from build123d import *

# Parameters (mm, degrees)
SKETCH_2_W          = 55
SKETCH_2_H          = 61
EXTRUDE_1_DEPTH     = 3
SKETCH_3_R          = 1.6
CUT_EXTRUDE_1_DEPTH = 3
FILLET_1_R          = 5
CUT_EXTRUDE_2_DEPTH = 3
FILLET_2_R          = 2


with BuildPart() as part:
    # 草图2 → 凸台-拉伸1 (new body)
    with BuildSketch(Plane(origin=(0, 0, 0), x_dir=(0, 0, -1), z_dir=(1, 0, 0))):
        with Locations((27.5, 30.5)):
            Rectangle(SKETCH_2_W, SKETCH_2_H)
    extrude(amount=EXTRUDE_1_DEPTH)

    # 草图3 → 切除-拉伸1 (cut)
    with BuildSketch(Plane.ZY):
        with Locations((-5, 56)):
            Circle(SKETCH_3_R)
        with Locations((-5, 37.5)):
            Circle(SKETCH_3_R)
        with Locations((-50, 56)):
            Circle(SKETCH_3_R)
        with Locations((-50, 37.5)):
            Circle(SKETCH_3_R)
        with Locations((-37.5, 3)):
            Circle(SKETCH_3_R)
        with Locations((-17.5, 3)):
            Circle(SKETCH_3_R)
    extrude(amount=-CUT_EXTRUDE_1_DEPTH, mode=Mode.SUBTRACT)

    # 圆角1
    fillet_1_edges = [part.edges().sort_by_distance(p)[0] for p in [
        (1.5, 61, 0),
        (1.5, 61, -55),
        (1.5, 0, -55),
        (1.5, 0, 0),
    ]]
    fillet(fillet_1_edges, radius=FILLET_1_R)

    # 草图4 → 切除-拉伸2 (cut)
    with BuildSketch(Plane.ZY):
        Polygon((-39.417495765, 57), (-27.5, 33), (-15.582504235, 57), align=None)
        Polygon((-45, 57), (-45, 33), (-33.082504235, 33), align=None)
        Polygon((-21.917495765, 33), (-10, 57), (-10, 33), align=None)
        Polygon((-10, 28), (-21.917495765, 28), (-10, 4), (-4, 4), (-4, 28), align=None)
        Polygon((-37.679527633, 7.5), (-27.5, 28), (-17.320472367, 7.5), align=None)
        Polygon((-45, 28), (-33.082504235, 28), (-45, 4), (-51, 4), (-51, 28), align=None)
    extrude(amount=-CUT_EXTRUDE_2_DEPTH, mode=Mode.SUBTRACT)

    # 圆角2
    fillet_2_edges = [part.edges().sort_by_distance(p)[0] for p in [
        (1.5, 57, -45),
        (1.5, 33, -33.082504235),
        (1.5, 33, -45),
        (1.5, 57, -39.417495765),
        (1.5, 57, -15.582504235),
        (1.5, 33, -27.5),
        (1.5, 28, -27.5),
        (1.5, 7.5, -17.320472367),
        (1.5, 7.5, -37.679527633),
        (1.5, 28, -4),
        (1.5, 4, -4),
        (1.5, 4, -10),
        (1.5, 28, -21.917495765),
        (1.5, 4, -51),
        (1.5, 28, -51),
        (1.5, 28, -33.082504235),
        (1.5, 4, -45),
        (1.5, 33, -10),
        (1.5, 33, -21.917495765),
        (1.5, 57, -10),
    ]]
    fillet(fillet_2_edges, radius=FILLET_2_R)


solid = part.part
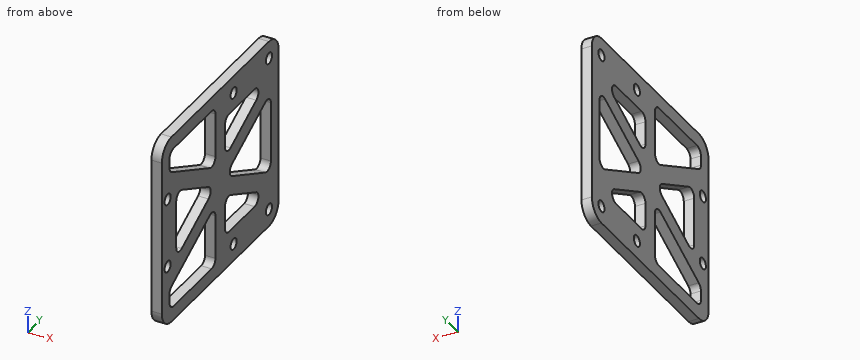
Check sheet for the modelled part. Datum: model origin and axes. Units: mm. Round coordinates to 2 decimals unless told otherwise and drop trailing zeros. Loops run counter-clockwise (first coordinate to the right, second up) from the corner with the lowest first, then second, coordinate; pieces in that order, holes last. Notation, with made-up numbers: M 48.5,14.25 L 87.5,14.25 A8 cw 87.5,27.25 Z; hole C -33.75,15.25 d6. An arc over 180 degrees is marked long. One line per item, written item: value.
(1) Sectioned sample at B-B, the plane y = 46. Record the cut outline in (x, z).
Computed values:
outline: M 0,-55 L 3,-55 L 3,-45 L 0,-45 Z; M 0,-39.54 L 3,-39.54 L 3,-33.96 L 0,-33.96 Z; M 0,-21.04 L 3,-21.04 L 3,-15.46 L 0,-15.46 Z; M 0,-10 L 3,-10 L 3,0 L 0,0 Z
(2) Sectioned sample at C-C, the plane x = 1.5. Count the separate pieces of the cut face and the enclosed holes in it, then the cut area to 3 significant figures.
Computed values:
separate pieces: 1
enclosed holes: 12
area: 1,990 mm^2
(3) Sectioned sample at D-D, the plane y = 34. Record the cut outline in (x, z), then the cut area to 3 significant figures.
Computed values:
outline: M 0,-55 L 3,-55 L 3,-44.73 L 0,-44.73 Z; M 0,-34.58 L 3,-34.58 L 3,-20.42 L 0,-20.42 Z; M 0,-10.27 L 3,-10.27 L 3,0 L 0,0 Z
area: 104 mm^2
(4) Sectioned sample at A-A, the plane y = 3. Record the cut outline in (x, z), then the cut area to 3 significant figures.
Computed values:
outline: M 0,-54.58 L 3,-54.58 L 3,-39.1 L 0,-39.1 Z; M 0,-35.9 L 3,-35.9 L 3,-19.1 L 0,-19.1 Z; M 0,-15.9 L 3,-15.9 L 3,-0.42 L 0,-0.42 Z
area: 143 mm^2
(5) Thickness scan on line 1 (Z direction, x = 2.3, y = 26); line 2 (Z direction, x = 0.8, y = 50); line 3 (Y direction, x = 2.35, z = -13). Record the ranges inside material, lowest first.
Computed values:
line 1: z = -55 to -51, -34.31 to -20.69, -4 to 0
line 2: z = -55 to -44.29, -41.71 to -35.94, -19.06 to -13.29, -10.71 to 0
line 3: y = 0 to 10.04, 28 to 33, 50.21 to 61
